Drawing for the job (mm, zero at the part's lowest x, y, z). A direction names the side the tool comes from. Round coordinates to 2 decimals unless told otherwise and drop trailing zeros. Loops run counter-clockwise (first coordinate to the right, second up) from the corner with the lowest first, then second, coordinate; pieces in that order, holes last. Notation, with made-up numbers: (35.25, 50.25) -> (60.25, 50.25) arc R7 ccw to (60.25, 58.25) -> close; hole circle Ø4 at (51.25, 87). An arc over 180 degrees is marked (long way). Put each result on its own line as item: value. Start each with the question number.
Item 1: Pull direction X, two halves, no side cores. Call the marked faces 3 and 4: +X half, -X half, draft (parallel to the pull), parting line (faces both ways), or undercut.
Item 2: Cut at B-B, the plane x = 38. List the corners of the cut face in (y, z), plus the area to 3 significant figures.
Item 3: Drill centre lines: probe 1 along X at (y, z) = (8, 7.25); probe 2 along Y at (x, z) = (8, 7); probe 3 along Y at (x, z) = (25, 9.25). Where is each one in solid material? Low to high. Write a range as [from, to].
Item 4: Cut at C-C, the plane z = 4.75. List the corners of the cut face in (x, y), plus the area to 3 significant figures.
Item 5: Cut at D-D, the plane y = 4.75. List the corners of the cut face in (x, z), plus the area to 3 significant figures.
Item 6: Cut at A-A, the plane y = 8. List the corners of the cut face in (x, z), plus the area to 3 significant figures.
Item 7: Tool access for the marked faces 1 and 2: list every direction of +Z, -Z, +X, -X, +Y, -Y with a clear straight run to the whole face (end or side of a thin tool).
Item 8: Flat gauge pins, fed straight in: pin 1 Ø1.5 at (y, z) = (12, 5.5) entering from +X; pin 2 Ø1 at (x, z) = (30, 6) entering from +Y; pin 3 Ø6.5 at (x, y) = (8, 8) entering from -Z. Where does each tip first touch, or does it go through?
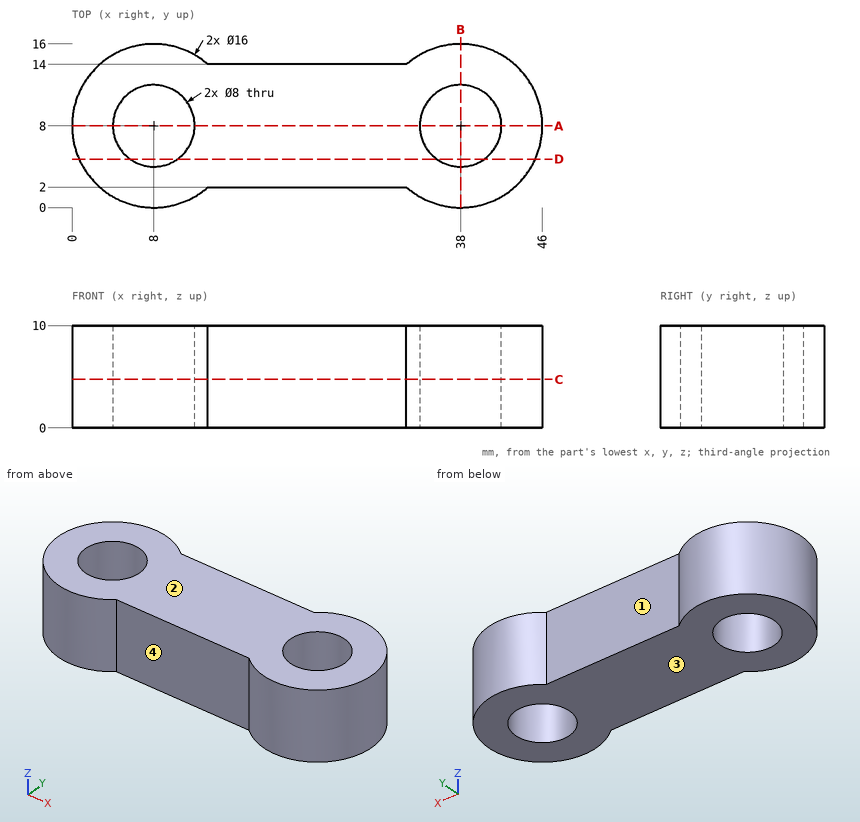
Reply:
1. face 3: draft
1. face 4: undercut
2. outline: (0, 0) -> (4, 0) -> (4, 10) -> (0, 10) -> close; (12, 0) -> (16, 0) -> (16, 10) -> (12, 10) -> close
2. area: 80.0 mm^2
3. probe 1: x = [0, 4], [12, 34], [42, 46]
3. probe 2: y = [0, 4], [12, 16]
3. probe 3: y = [2, 14]
4. outline: (13.29, 2) -> (32.71, 2) arc R8 ccw (long way) to (32.71, 14) -> (13.29, 14) arc R8 ccw (long way) to start; hole circle Ø8 at (8, 8); hole circle Ø8 at (38, 8)
4. area: 490 mm^2
5. outline: (0.69, 0) -> (5.67, 0) -> (5.67, 10) -> (0.69, 10) -> close; (10.33, 0) -> (35.67, 0) -> (35.67, 10) -> (10.33, 10) -> close; (40.33, 0) -> (45.31, 0) -> (45.31, 10) -> (40.33, 10) -> close
5. area: 353 mm^2
6. outline: (0, 0) -> (4, 0) -> (4, 10) -> (0, 10) -> close; (12, 0) -> (34, 0) -> (34, 10) -> (12, 10) -> close; (42, 0) -> (46, 0) -> (46, 10) -> (42, 10) -> close
6. area: 300 mm^2
7. face 1: +Z, -Z, +Y
7. face 2: +Z, +X, -X, +Y, -Y
8. pin 1: stops at x = 45.31
8. pin 2: stops at y = 14
8. pin 3: passes through
